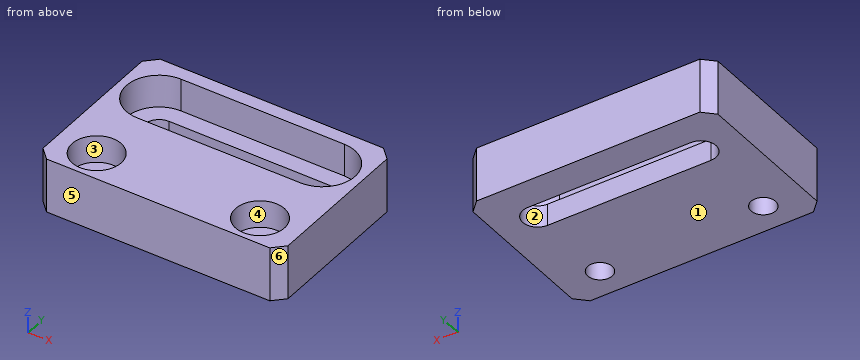
```python
from build123d import *

# Parameters (mm, degrees)
SKETCH1_W           = 45
SKETCH1_H           = 31
BOSS_EXTRUDE1_DEPTH = 10
CUT_EXTRUDE1_DEPTH  = 13
SKETCH3_R           = 4.5
CUT_EXTRUDE2_DEPTH  = 5
SKETCH4_R           = 2.25
CUT_EXTRUDE3_DEPTH  = 14
CHAMFER1_SIZE       = 2
CUT_EXTRUDE4_DEPTH  = 6


with BuildPart() as part:
    # Sketch1 → Boss-Extrude1 (new body)
    with BuildSketch(Plane.XY):
        Rectangle(SKETCH1_W, SKETCH1_H)
    extrude(amount=BOSS_EXTRUDE1_DEPTH)

    # Sketch2 → Cut-Extrude1 (cut)
    with BuildSketch(Plane.XY.offset(10)):
        with BuildLine():
            Line((-15, 9.75), (15, 9.75))
            ThreePointArc((15, 9.75), (17.75, 7), (15, 4.25))
            Line((15, 4.25), (-15, 4.25))
            ThreePointArc((-15, 4.25), (-17.75, 7), (-15, 9.75))
        make_face()
    extrude(amount=-CUT_EXTRUDE1_DEPTH, mode=Mode.SUBTRACT)

    # Sketch3 → Cut-Extrude2 (cut)
    with BuildSketch(Plane.XY.offset(10)):
        with Locations((-15, -10)):
            Circle(SKETCH3_R)
        with Locations(Location((15, -10, 0), (0, 0, 180))):
            Circle(SKETCH3_R)
    extrude(amount=-CUT_EXTRUDE2_DEPTH, mode=Mode.SUBTRACT)

    # Sketch4 → Cut-Extrude3 (cut)
    with BuildSketch(Plane.XY.offset(10)):
        with Locations((-15, -10)):
            Circle(SKETCH4_R)
        with Locations((15, -10)):
            Circle(SKETCH4_R)
    extrude(amount=-CUT_EXTRUDE3_DEPTH, mode=Mode.SUBTRACT)

    # Chamfer1
    chamfer1_edges = [part.edges().sort_by_distance(p)[0] for p in [
        (22.5, -15.5, 5),
        (-22.5, -15.5, 5),
        (-22.5, 15.5, 5),
        (22.5, 15.5, 5),
    ]]
    chamfer(chamfer1_edges, length=CHAMFER1_SIZE)

    # Sketch5 → Cut-Extrude4 (cut)
    with BuildSketch(Plane.XY.offset(10)):
        with BuildLine():
            Line((-15, 13), (15, 13))
            ThreePointArc((15, 13), (21, 7), (15, 1))
            Line((15, 1), (-15, 1))
            ThreePointArc((-15, 1), (-21, 7), (-15, 13))
        make_face()
    extrude(amount=-CUT_EXTRUDE4_DEPTH, mode=Mode.SUBTRACT)


solid = part.part
```
Input: part model. Units: mm. Frame: model coordinates. Face numbers are marked on the shaded views. A direction names the side the tool comes from. Give positions to 0.01 mm unless a question says otherwise; leave off trailing zeros. Order: outer loops, then holes, each group sorted by start corner. A loop starts at its lowest first (then second) coordinate and runs counter-clockwise, first axis right, second up. Notation, with made-up numbers: (21, -28.5) - (49, -28.5) arc R16 ccw to (49, -1.5) - close; hole circle Ø6 at (57.25, 58.5). An arc over 180 degrees is marked (long way). One line per item, written item: value.
1. Reachability of the marked faces 1, 2 and 3 from +Z, -Z, +X, -X, +Y, -Y: full face, straight path, thin tool, end or side. Return the list, or none.
Determined:
face 1: -Z, +X, -X, +Y, -Y
face 2: +Z, -Z
face 3: +Z
2. Cut plane C-C, the plane x = 8.5. Output: boundary loops of the cut face in (y, z).
Determined:
outline: (-15.5, 0) - (4.25, 0) - (4.25, 4) - (1, 4) - (1, 10) - (-15.5, 10) - close; (9.75, 0) - (15.5, 0) - (15.5, 10) - (13, 10) - (13, 4) - (9.75, 4) - close
3. Cut plane B-B, the plane z = 7.25. Output: boundary loops of the cut face in (x, y), and give its area (3 significant figures).
Determined:
outline: (-22.5, -13.5) - (-20.5, -15.5) - (20.5, -15.5) - (22.5, -13.5) - (22.5, 13.5) - (20.5, 15.5) - (-20.5, 15.5) - (-22.5, 13.5) - close; hole circle Ø9 at (-15, -10); hole (-15, 1) - (15, 1) arc R6 ccw to (15, 13) - (-15, 13) arc R6 ccw to start; hole circle Ø9 at (15, -10)
area: 787 mm2
4. Pin query (flat end, axial travel): pin 1 Ø4 at (x, y) = (-10.5, 6) entering from +Z; pin 2 Ø2.5 at (x, y) = (14.5, -11.5) entering from +Z; pin 3 Ø4 at (x, y) = (15, -10) entering from +Z. Return the tip coordinate at first contact, or that it passes through.
Determined:
pin 1: z = 4
pin 2: z = 5
pin 3: through
5. Cut plane A-A, the plane y = 7. Output: boundary loops of the cut face in (x, z).
Determined:
outline: (-22.5, 0) - (-17.75, 0) - (-17.75, 4) - (-21, 4) - (-21, 10) - (-22.5, 10) - close; (17.75, 0) - (22.5, 0) - (22.5, 10) - (21, 10) - (21, 4) - (17.75, 4) - close
6. Draft query along X for the marked faces 4, 5 and 6. Return one class per face: released by +X, released by -X, zero draft, split by the parting line, or undercut.
Determined:
face 4: undercut
face 5: zero draft
face 6: released by +X
7. Line query: probe 1 along Y at (x, z) = (15, 9.75); probe 2 along Y at (x, z) = (15, 3.45); probe 3 along Y at (x, z) = (3.5, 2.5). Output: solid intervals per line, ascending.
Determined:
probe 1: -15.5 to -14.5, -5.5 to 1, 13 to 15.5
probe 2: -15.5 to -12.25, -7.75 to 4.25, 9.75 to 15.5
probe 3: -15.5 to 4.25, 9.75 to 15.5
8. Cut plane D-D, the plane x = -16.5. Output: boundary loops of the cut face in (y, z), and give its area (3 significant figures).
Determined:
outline: (-15.5, 0) - (-11.68, 0) - (-11.68, 5) - (-14.24, 5) - (-14.24, 10) - (-15.5, 10) - close; (-8.32, 0) - (4.7, 0) - (4.7, 4) - (1.19, 4) - (1.19, 10) - (-5.76, 10) - (-5.76, 5) - (-8.32, 5) - close; (9.3, 0) - (15.5, 0) - (15.5, 10) - (12.81, 10) - (12.81, 4) - (9.3, 4) - close
area: 163 mm2
